Check sheet for the modelled part. Datum: model origin and axes. Units: mm. Face numbers are marked on the shaded views. A direction names the side the tool comes from. Round coordinates to 2 decimals unless told otherwise and drop trailing zeros. Order: outer loops, then holes, each group sorted by start corner. A loop starts at its lowest first (then second) coordinate and runs counter-clockwise, first axis right, second up. Notation, with made-up numbers: (55.5, 15) -> (81.5, 15) arc R11 cw to (81.5, 33) -> close; hole circle Ø2 at (64, 51.5). An arc over 180 degrees is marked (long way). Answer in a Markdown table with one row per item. Add a question column.
1. Draft check along X on the marked faces 1, 2 and 3. Enter one of: +X half, -X half, draft (parallel to the pull), parting line (faces both ways), or undercut.
2. Depth check by flat-ended pin: P1, Ø10, axis at x = -158, y = 16, coming from the -Z side; P2, Ø7.5, axis at x = 185, z = 0, coming from the -Y side; P3, Ø7, axis at x = -130.81, z = -130.81, coming from the -Y side. Enter the tip coordinate at first touch or a pass-through.
3. Sectioned sample at A-A, the plane y = 54. Record the boundary of the cut face in (x, z), then the cut area to 3 significant figures.
4. Material ranges on L1, parallel to X at y = 9, z = 0; L2, parallel to X at y = 54, z = -11.5; L3, parallel to X at y = 81, z = -2, recorded low to high. Write a range as from..to.
5. Access from +Z, -Z, +X, -X, +Y, -Y to the whole of each face (thin tool, end or side, straight path). Record for the marked faces 4 and 5.
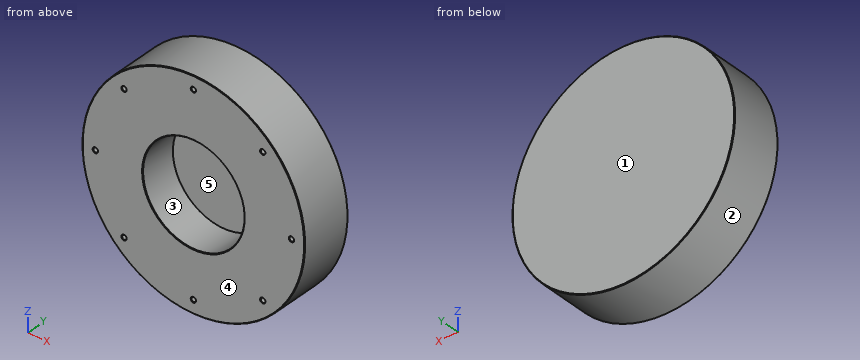
```python
from build123d import *

# Parameters (mm, degrees)
SKETCH_1_R               = 210
SKETCH_1_R_2             = 95.82
EXTRUDE_1_DEPTH          = 100
SKETCH_5_R               = 150
EXTRUDE_4_DEPTH          = 30
PATTERN_CIRCULAR_1_COUNT = 8
CHAMFER_1_SIZE           = 1


with BuildPart() as part:
    # 草图1 → 凸台-拉伸1 (new body)
    with BuildSketch(Plane(origin=(0, 0, 0), x_dir=(1, 0, 0), z_dir=(0, 1, 0))):
        with Locations(Location((0, 0, 0), (0, 0, 270))):
            Circle(SKETCH_1_R)
        with Locations(Location((0, 0, 0), (0, 0, 270))):
            Circle(SKETCH_1_R_2, mode=Mode.SUBTRACT)
    extrude(amount=EXTRUDE_1_DEPTH)

    # 草图5 → 凸台-拉伸4 (add)
    with BuildSketch(Plane(origin=(0, 100, 0), x_dir=(1, 0, 0), z_dir=(0, 1, 0))):
        Circle(SKETCH_5_R)
    extrude(amount=-EXTRUDE_4_DEPTH)

    # 草图8 → M10 螺纹孔1 (revolve, cut)
    with BuildSketch(Plane(origin=(185, 0, 0), x_dir=(0, 0, -1), z_dir=(1, 0, 0))):
        Polygon((0, 0), (0, 30.053657631), (4.25, 27.5), (4.25, 0.775), (5.025, 0), align=None)
    hole_wizard_m10_1 = revolve(axis=Axis((185, -6.35, 0), (0, 1, 0)), mode=Mode.SUBTRACT)

    # 阵列(圆周)1: M10 螺纹孔1 ×8 about axis
    pattern_circular_1_axis = Axis((0, 0, 0), (0, 1, 0))
    for i in range(1, PATTERN_CIRCULAR_1_COUNT):
        add(hole_wizard_m10_1.rotate(pattern_circular_1_axis, i * 360 / PATTERN_CIRCULAR_1_COUNT), mode=Mode.SUBTRACT)

    # 倒角1
    chamfer_1_edges = [part.edges().sort_by_distance(p)[0] for p in [
        (0, 0, -210),
        (0, 100, -210),
        (0, 0, -95.82),
    ]]
    chamfer(chamfer_1_edges, length=CHAMFER_1_SIZE)


solid = part.part
```
Answer key:
| question | item | result |
|---|---|---|
| 1 | face 1 | draft |
| 1 | face 2 | parting line |
| 1 | face 3 | undercut |
| 2 | P1 | stops at z = -143.84 |
| 2 | P2 | stops at y = 27.8 |
| 2 | P3 | stops at y = 27.95 |
| 3 | outline | circle Ø420 at (0, 0); hole circle Ø191.64 at (0, 0) |
| 3 | area | 110,000 mm² |
| 4 | L1 | x = -210..-189.25, -180.75..-95.82, 95.82..180.75, 189.25..210 |
| 4 | L2 | x = -209.68..-95.13, 95.13..209.68 |
| 4 | L3 | x = -209.99..209.99 |
| 5 | face 4 | +Z, -Z, +X, -X, -Y |
| 5 | face 5 | -Y |
